```python
from build123d import *

# Parameters (mm, degrees)
SKETCH1_W           = 170
SKETCH1_H           = 350
SKETCH1_R           = 60
SKETCH1_R_2         = 22.5
BOSS_EXTRUDE1_DEPTH = 3


with BuildPart() as part:
    # Sketch1 → Boss-Extrude1 (new body)
    with BuildSketch(Plane.XY):
        with Locations((85, 175)):
            Rectangle(SKETCH1_W, SKETCH1_H)
        with Locations((85, 210)):
            Circle(SKETCH1_R, mode=Mode.SUBTRACT)
        with Locations((85, 60)):
            Circle(SKETCH1_R_2, mode=Mode.SUBTRACT)
    extrude(amount=BOSS_EXTRUDE1_DEPTH)


solid = part.part
```
Verification items for the finished model (mm, model axes). Give positions to 0.01 mm unless a question says otherwise; leave off trailing zeros. Write each loop counter-clockwise with the first axis right and the second up, starting at its lowest first coordinate (ties: lowest second). Pieces come first, ordered by that corner, then holes. Notation, with made-up numbers: M 29.5,23 L 76.5,23 A20 cw 76.5,55 Z; hole C 31,-2 d3. An arc over 180 degrees is marked long. One line per question, with ' | ' between items.
1) Section check D-D on y = 60. Enter the section's corners in (x, z).
Result:
outline: M 0,0 L 62.5,0 L 62.5,3 L 0,3 Z; M 107.5,0 L 170,0 L 170,3 L 107.5,3 Z
2) Section check C-C on x = 99. Enter the section's corners in (y, z).
Result:
outline: M 0,0 L 42.39,0 L 42.39,3 L 0,3 Z; M 77.61,0 L 151.66,0 L 151.66,3 L 77.61,3 Z; M 268.34,0 L 350,0 L 350,3 L 268.34,3 Z
3) Thickness scan on line 1 along Y through (x, z) = (85, 0.9); line 2 along Y through (x, z) = (103, 2.45); line 3 along X through (y, z) = (190, 2.2). Record the ranges inside material, lowest first. Write a range as [from, to].
Result:
line 1: y = [0, 37.5], [82.5, 150], [270, 350] | line 2: y = [0, 46.5], [73.5, 152.76], [267.24, 350] | line 3: x = [0, 28.43], [141.57, 170]
4) Section check B-B on z = 0.8. Enter the section's corners in (x, y).
Result:
outline: M 0,0 L 170,0 L 170,350 L 0,350 Z; hole C 85,210 d120; hole C 85,60 d45
5) Mould release check, pull along X, two halves, no side actions. Record for faces 1 (the flat face through (84, 139, 0)), 2 (the cylindrical face through (40.778, 250.551, 1.479)), 3 (the cylindrical face through (62.52, 60.99, 1.48)): released by +X, released by -X, zero draft, split by the parting line, or undercut.
Result:
face 1: zero draft | face 2: undercut | face 3: undercut
6) Section check A-A on y = 210. Enter the section's corners in (x, z), plus the area to 3 significant figures.
Result:
outline: M 0,0 L 25,0 L 25,3 L 0,3 Z; M 145,0 L 170,0 L 170,3 L 145,3 Z | area: 150 mm2
